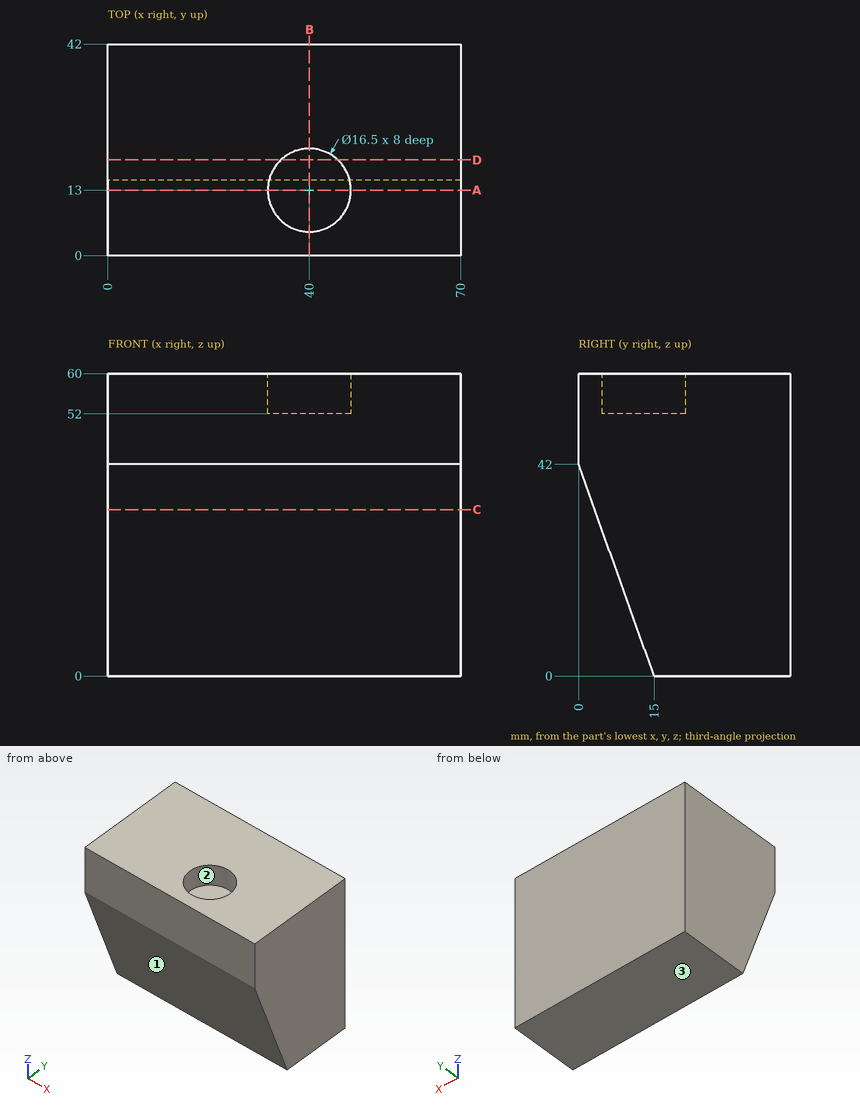
Can you work these out from the drawing? Everything is in mm from the part's minimum corner. Give positions to 0.01 mm unless a question says otherwise; leave off trailing zeros. Order: outer loops, then holes, each group sorted by start corner. A loop starts at its lowest first (then second) coordinate and runs counter-clockwise, first axis right, second up. Notation, with made-up numbers: (25, -21.75) -> (83, -21.75) arc R14 ccw to (83, -17.75) -> close; hole circle Ø5 at (-11.75, 27.5). An arc over 180 degrees is marked (long way). Return JSON: item names as keys, results as strings.
1. For pin 1 Ø13 at (x, y) = (40, 13) entering from +Z; pin 2 Ø4 at (x, z) = (37, 23.5) entering from -Y; pin 3 Ø3 at (x, z) = (56.5, 17) entering from -Y, each with a flat end and sliding along its axis, tell me the tip position at first contact or that it passes through.
Answer list:
{"pin 1": "stops at z = 52", "pin 2": "stops at y = 5.89", "pin 3": "stops at y = 8.39"}
2. Imagine slicing it at A-A on y = 13. List the corners of the cut face in (x, z) for me.
Answer list:
{"outline": "(0, 5.6) -> (70, 5.6) -> (70, 60) -> (48.25, 60) -> (48.25, 52) -> (31.75, 52) -> (31.75, 60) -> (0, 60) -> close"}
3. Imagine slicing it at D-D on y = 19. List the corners of the cut face in (x, z) for me, then the cut area to 3 significant figures.
Answer list:
{"outline": "(0, 0) -> (70, 0) -> (70, 60) -> (45.66, 60) -> (45.66, 52) -> (34.34, 52) -> (34.34, 60) -> (0, 60) -> close", "area": "4,110 mm2"}
4. Imagine slicing it at C-C on z = 33. List the corners of the cut face in (x, y) for me, then the cut area to 4 significant figures.
Answer list:
{"outline": "(0, 3.21) -> (70, 3.21) -> (70, 42) -> (0, 42) -> close", "area": "2,715 mm2"}
5. Imagine slicing it at B-B on x = 40. List the corners of the cut face in (y, z) for me.
Answer list:
{"outline": "(0, 42) -> (15, 0) -> (42, 0) -> (42, 60) -> (21.25, 60) -> (21.25, 52) -> (4.75, 52) -> (4.75, 60) -> (0, 60) -> close"}
6. I need wall thicknesses on line 1 (Y direction, x = 40, z = 54.25); line 2 (Y direction, x = 43, z = 38); line 3 (Y direction, x = 63.5, z = 27). Which ranges of each line are inside material? Lowest first, please. Write a range as from..to.
Answer list:
{"line 1": "y = 0..4.75, 21.25..42", "line 2": "y = 1.43..42", "line 3": "y = 5.36..42"}
7. Thinking about a two-plate mould opening in Y: for the marked faces 1, 2 and 3, which applies, pulls with the +Y half, pulls with the -Y half, needs draft (parallel to the pull), parting line crosses it, or undercut?
Answer list:
{"face 1": "pulls with the -Y half", "face 2": "undercut", "face 3": "needs draft"}
